Read the model definition and answer for the solid it produces. Units are mm, in the model's axes. A direction names the side the tool comes from. Coordinates: 2 decimals unless noted, no trailing zeros. Loops run counter-clockwise (first coordinate to the right, second up) from the corner with the lowest first, then second, coordinate; pieces in that order, holes last. Notation, with made-up numbers: (27.5, -8.5) -> (74.5, -8.5) arc R25 ccw to (74.5, 12.5) -> close; hole circle Ø3 at (67.5, 48). An arc over 180 degrees is marked (long way). Answer as a JSON object with one key per item and string values. Group by question number.
1) Determine the mould class of faces 6 (the face through (-135, 15, 0)), 7 (the face through (-100, -16, 0)), 8 (the face through (-58, -16, 0)), 9 (the face through (-66.55, 34.07, -10.65)) for opening direction X: released by +X, released by -X, zero draft, split by the parting line, or undercut.
2) Flat-ended cylindrical pins translate along their axes: P1, Ø10, axis at x = -99.5, z = -13, coming from the -Y side; P2, Ø18.5, axis at x = -59, y = -14.5, coming from the -Z side; P3, Ø8, axis at x = -92, z = -9, coming from the +Y side. Find the tip coordinate at first contact, or state that the pin passes through.
3) Section C-C, the plane y = 41.5 is taken. Give the vertices of the cut face in (x, z).
4) Section D-D, the plane z = -1.5 is taken. Give the vertices of the cut face in (x, y) (3 decimals), plus the area to 3 significant figures.
5) Consider probe 1 along Z at (x, y) = (-81.5, -0.5); probe 2 along Y at (x, z) = (-85, 22); probe 3 along Z at (x, y) = (-108, 46.5). Determine where each line is inside the solid, lowest interval first. Write a range as [from, to].
6) Section B-B, the plane x = -24.5 is taken. Give the vertices of the cut face in (y, z), plus the area to 3 significant figures.
7) Which of the six approach directions +Z, -Z, +X, -X, +Y, -Y give full straight-line access (tool end or side, diameter ignored) to faces 1 (the face through (-67, 0, 20)), 2 (the face through (-66.555, 33.559, 10.353)), 3 (the face through (-67, 26, 30)), 4 (the face through (-67, 0, -19)), 5 (the face through (-44, -16, 0))?
8) Section A-A, the plane y = -15 is taken. Give the vertices of the cut face in (x, z).
from build123d import *

# Parameters (mm, degrees)
V_BLOCK_BODY_DEPTH          = 135
UNDERSIDE_NOTCHES_CUT_DEPTH = 195


with BuildPart() as part:
    # V-Block Profile Sketch → V-Block Body (new body)
    with BuildSketch(Plane(origin=(0, 0, 0), x_dir=(0, 0, -1), z_dir=(1, 0, 0))):
        Polygon((-30, 52), (-30, 0), (-9, 0), (-9, -23), (9, -23), (9, 0), (30, 0), (30, 52), (21, 52), (0, 15.626933041), (-21, 52), align=None)
    extrude(amount=-V_BLOCK_BODY_DEPTH)

    # Underside Notches Sketch → Underside Notches Cut (cut)
    with BuildSketch(Plane.XY.offset(9)):
        Polygon((-135, -23), (-121, -9), (-107, -23), (-93, -9), (-79, -23), (-65, -9), (-51, -23), (-37, -9), (-7.657800388, -38.342199612), (-135, -44.429564146), align=None)
    extrude(amount=-UNDERSIDE_NOTCHES_CUT_DEPTH, mode=Mode.SUBTRACT)


solid = part.part
Determined:
{
 "1": {"face 6": "released by -X", "face 7": "undercut", "face 8": "undercut", "face 9": "zero draft"},
 "2": {"P1": "y = -18.5", "P2": "z = -9", "P3": "y = 38.14"},
 "3": {"outline": "(-135, -30) -> (0, -30) -> (0, -14.94) -> (-135, -14.94) -> close; (-135, 14.94) -> (0, 14.94) -> (0, 30) -> (-135, 30) -> close"},
 "4": {"outline": "(-135, -23) -> (-121, -9) -> (-107, -23) -> (-93, -9) -> (-79, -23) -> (-65, -9) -> (-51, -23) -> (-37, -9) -> (-23, -23) -> (0, -23) -> (0, 18.225) -> (-135, 18.225) -> close", "area": "4,780 mm²"},
 "5": {"probe 1": "[-9, 9]", "probe 2": "[0, 52]", "probe 3": "[-30, -17.82], [17.82, 30]"},
 "6": {"outline": "(-21.5, -9) -> (0, -9) -> (0, -30) -> (52, -30) -> (52, -21) -> (15.63, 0) -> (52, 21) -> (52, 30) -> (0, 30) -> (0, 9) -> (-21.5, 9) -> close", "area": "2,740 mm²"},
 "7": {"face 1": "+Z, +X, -X, -Y", "face 2": "+X, -X, +Y", "face 3": "+Z, +X, -X, +Y, -Y", "face 4": "-Z, +X, -X, -Y", "face 5": "+Z, -Z, -Y"},
 "8": {"outline": "(-135, -9) -> (-127, -9) -> (-127, 9) -> (-135, 9) -> close; (-115, -9) -> (-99, -9) -> (-99, 9) -> (-115, 9) -> close; (-87, -9) -> (-71, -9) -> (-71, 9) -> (-87, 9) -> close; (-59, -9) -> (-43, -9) -> (-43, 9) -> (-59, 9) -> close; (-31, -9) -> (0, -9) -> (0, 9) -> (-31, 9) -> close"}
}
